from build123d import *

# Parameters (mm, degrees)
SKETCH_1_R               = 60
SKETCH_1_R_2             = 17.75
EXTRUDE_1_DEPTH          = 42.5
PATTERN_CIRCULAR_1_COUNT = 8
PATTERN_CIRCULAR_2_COUNT = 4
SKETCH_6_R               = 5
CUT_EXTRUDE_1_DEPTH      = 90


with BuildPart() as part:
    # 草图1 → 凸台-拉伸1 (new, symmetric)
    with BuildSketch(Plane.XY):
        Circle(SKETCH_1_R)
        Circle(SKETCH_1_R_2, mode=Mode.SUBTRACT)
    extrude(amount=EXTRUDE_1_DEPTH, both=True)

    # 草图3 → M6x1.0 螺纹孔1 (revolve, cut)
    with BuildSketch(Plane(origin=(0, 50, 42.5), x_dir=(0, -1, 0), z_dir=(1, 0, 0))):
        Polygon((0, 0), (0, 16.502151548), (2.5, 15), (2.5, 0), align=None)
    m6x1_0_1 = revolve(axis=Axis((0, 50, 48.85), (0, 0, -1)), mode=Mode.SUBTRACT)

    # 阵列(圆周)1: M6x1.0 螺纹孔1 ×8 about axis
    pattern_circular_1_axis = Axis((0, 0, 0), (0, 0, 1))
    for i in range(1, PATTERN_CIRCULAR_1_COUNT):
        add(m6x1_0_1.rotate(pattern_circular_1_axis, i * 360 / PATTERN_CIRCULAR_1_COUNT), mode=Mode.SUBTRACT)

    # 草图5 → M4x0.7 螺纹孔1 (revolve, cut)
    with BuildSketch(Plane(origin=(-36, 0, -42.5), x_dir=(0, 1, 0), z_dir=(1, 0, 0))):
        Polygon((0, 0), (0, 11.091420021), (1.65, 10.1), (1.65, 0), align=None)
    m4x0_7_1 = revolve(axis=Axis((-36, 0, -48.85), (0, 0, 1)), mode=Mode.SUBTRACT)

    # 阵列(圆周)2: M4x0.7 螺纹孔1 ×4 about axis
    pattern_circular_2_axis = Axis((0, 0, 0), (0, 0, 1))
    for i in range(1, PATTERN_CIRCULAR_2_COUNT):
        add(m4x0_7_1.rotate(pattern_circular_2_axis, i * 360 / PATTERN_CIRCULAR_2_COUNT), mode=Mode.SUBTRACT)

    # 草图6 → 切除-拉伸1 (cut, symmetric)
    with BuildSketch(Plane(origin=(0, 0, 0), x_dir=(-0.7071067811865438, -0.7071067811865512, 0), z_dir=(0.7071067811865512, -0.7071067811865438, 0))):
        with Locations(Location((0, 0, 0), (0, 0, 180))):
            Circle(SKETCH_6_R)
    extrude(amount=CUT_EXTRUDE_1_DEPTH, both=True, mode=Mode.SUBTRACT)


solid = part.part
Here's how the part is built. I have some questions about the finished solid (model axes, mm). A direction names the side the tool comes from. Round coordinates to 2 decimals unless told otherwise and drop trailing zeros. Loops run counter-clockwise (first coordinate to the right, second up) from the corner with the lowest first, then second, coordinate; pieces in that order, holes last. Notation, with made-up numbers: M 52.5,65.25 L 99.5,65.25 A19 cw 99.5,74.25 Z; hole C 7.5,2 d9. An arc over 180 degrees is marked long. Write each question's results on one line, items separated by ' | '. Start each with the question number.
(1) On a 3-axis mill with a long thin cutter (end or side, diameter ignored), from which of +Z, -Z, +X, -X, +Y, -Y can I reach the whole of each face in a straight line? I mean faces 1 (the cylindrical face through (37.39, -0.89, -37.52)), 2 (the cylindrical face through (47.69, -0.96, 35.11)), 3 (the cylindrical face through (30.71, -24.18, -1.92)). Say none if no direction works.
(2) Will these pins go through, and if not, where does the flat tip stop? P1, Ø3, axis at x = -35.36, y = 35.36, coming from the +Z side; P2, Ø2.5, axis at x = 0, y = -36, coming from the -Z side; P3, Ø10, axis at x = 21.5, z = 32, coming from the +Y side.
(3) I want a section at A-A (z = 31). State how many separate pieces and enclosed holes the cut face has, then the cut area to 3 significant figures.
(4) If I drill on probe 1 along X at (y, z) = (-3, -35.5); probe 2 along Y at (x, z) = (1.5, -27); probe 3 along X at (y, z) = (8, -30), over which ranges is the centre line in solid material (lowest first)? Write a range as from..to.
(5) Thinking about a two-plate mould opening in X: for faces 4 (the flat face through (12, 14, -42.5)), 5 (the cylindrical face through (-23.76, 30.29, -1.92)), 6 (the cylindrical face through (55.425, -22.98, 0.595)), which applies, pulls with the +X half, pulls with the -X half, needs draft (parallel to the pull), parting line crosses it, or undercut?
(6) I want a section at B-B (z = -26). Please give me the cut outline in (x, y), then the cut area to 3 significant figures.
Solved:
1) face 1: -Z | face 2: +Z | face 3: none
2) P1: stops at z = 26.9 | P2: stops at z = -32.16 | P3: stops at y = 57.69
3) separate pieces: 1 | enclosed holes: 9 | area: 10,200 mm²
4) probe 1: x = -59.92..-17.49, 17.49..59.92 | probe 2: y = -59.98..-17.69, 17.69..59.98 | probe 3: x = -59.46..-15.84, 15.84..59.46
5) face 4: needs draft | face 5: undercut | face 6: parting line crosses it
6) outline: C 0,0 d120; hole C 0,0 d35.5 | area: 10,300 mm²
